```python
from build123d import *

# Parameters (mm, degrees)
BOSS_EXTRUDE1_DEPTH   = 210
SKETCH2_OUTSIDE_W     = 58.016
SKETCH2_OUTSIDE_H     = 56.16
SKETCH2_OUTSIDE_R     = 5
CUT_EXTRUDE1_DEPTH    = 8
SKETCH3_OUTSIDE_W     = 58.016
SKETCH3_OUTSIDE_H     = 56.16
SKETCH3_OUTSIDE_R     = 5
CUT_EXTRUDE2_DEPTH    = 8
M6_TAPPED_HOLE1_D     = 5
M5_TAPPED_HOLE1_D     = 4.2
M5_TAPPED_HOLE1_DEPTH = 12.4
M5_TAPPED_HOLE1_TIP   = 1.2618073
M5_TAPPED_HOLE2_D     = 4.2
M5_TAPPED_HOLE2_DEPTH = 12.4
M5_TAPPED_HOLE2_TIP   = 1.2618073
CHAMFER1_SIZE         = 0.3


with BuildPart() as part:
    # Sketch1 → Boss-Extrude1 (new body)
    with BuildSketch(Plane(origin=(0, 0, 0), x_dir=(1, 0, 0), z_dir=(0, 1, 0))):
        Polygon((6.92820323, 0), (3.464101615, 6), (-3.464101615, 6), (-6.92820323, 0), (-3.464101615, -6), (3.464101615, -6), align=None)
    extrude(amount=BOSS_EXTRUDE1_DEPTH)

    # Sketch2 outside → Cut-Extrude1 (cut)
    with BuildSketch(Plane(origin=(0, 210, 0), x_dir=(1, 0, 0), z_dir=(0, 1, 0))):
        Rectangle(SKETCH2_OUTSIDE_W, SKETCH2_OUTSIDE_H)
        with Locations(Location((0, 0, 0), (0, 0, 270))):
            Circle(SKETCH2_OUTSIDE_R, mode=Mode.SUBTRACT)
    extrude(amount=-CUT_EXTRUDE1_DEPTH, mode=Mode.SUBTRACT)

    # Sketch3 outside → Cut-Extrude2 (cut)
    with BuildSketch(Plane.XZ):
        Rectangle(SKETCH3_OUTSIDE_W, SKETCH3_OUTSIDE_H)
        with Locations(Location((0, 0, 0), (0, 0, 90))):
            Circle(SKETCH3_OUTSIDE_R, mode=Mode.SUBTRACT)
    extrude(amount=-CUT_EXTRUDE2_DEPTH, mode=Mode.SUBTRACT)

    # M6 Tapped Hole1 (through all)
    with Locations(Plane(origin=(0, 0, -6), x_dir=(-1, 0, 0), z_dir=(0, 0, -1))):
        with Locations((0, 140), (0, 70)):
            Hole(M6_TAPPED_HOLE1_D / 2)

    # M5 Tapped Hole1
    with Locations(Plane.XZ):
        with Locations((0, 0)):
            Hole(M5_TAPPED_HOLE1_D / 2, depth=M5_TAPPED_HOLE1_DEPTH)
            with Locations((0, 0, -(M5_TAPPED_HOLE1_DEPTH + M5_TAPPED_HOLE1_TIP / 2))):  # 118° drill point
                Cone(0, M5_TAPPED_HOLE1_D / 2, M5_TAPPED_HOLE1_TIP, mode=Mode.SUBTRACT)

    # M5 Tapped Hole2
    with Locations(Plane(origin=(0, 210, 0), x_dir=(-1, 0, 0), z_dir=(0, 1, 0))):
        with Locations((0, 0)):
            Hole(M5_TAPPED_HOLE2_D / 2, depth=M5_TAPPED_HOLE2_DEPTH)
            with Locations((0, 0, -(M5_TAPPED_HOLE2_DEPTH + M5_TAPPED_HOLE2_TIP / 2))):  # 118° drill point
                Cone(0, M5_TAPPED_HOLE2_D / 2, M5_TAPPED_HOLE2_TIP, mode=Mode.SUBTRACT)

    # Chamfer1
    chamfer1_edges = [part.edges().sort_by_distance(p)[0] for p in [
        (0, 210, -5),
        (0, 0, -5),
    ]]
    chamfer(chamfer1_edges, length=CHAMFER1_SIZE)


solid = part.part
```
The model under review builds one solid part; all positions refer to its coordinate system, in mm. A direction names the side the tool comes from. Round coordinates to 2 decimals unless told otherwise and drop trailing zeros. Order: outer loops, then holes, each group sorted by start corner. A loop starts at its lowest first (then second) coordinate and runs counter-clockwise, first axis right, second up. Notation, with made-up numbers: M -37,59 L 21,59 A24 ccw 21,95 Z; hole C 34,37.5 d11. An arc over 180 degrees is marked long. Use a Markdown table: item, result.
1) Consider section A-A (y = 70). Write out the cut boundary in (x, z).
Report:
| item | result |
|---|---|
| outline | M -6.93,0 L -3.46,-6 L -2.5,-6 L -2.5,6 L -3.46,6 Z; M 2.5,-6 L 3.46,-6 L 6.93,0 L 3.46,6 L 2.5,6 Z |
2) Tool access review of faces 1 (the face through (-4.88, 205.9, -1.08)), 2 (the face through (-5.172, 103.642, -3.042)), 3 (the face through (-2.003, 6.287, 0.631)): name each direction out of +Z, -Z, +X, -X, +Y, -Y from which nothing blocks a thin tool from reaching the whole face with its end or side.
Report:
| item | result |
|---|---|
| face 1 | +Y |
| face 2 | -Z, -X, +Y, -Y |
| face 3 | -Y |
3) Draft analysis for pull direction X (two halves, no side actions). For faces 4 (the face through (-0.33, 142.48, 0.08)), 5 (the face through (-1.1, 0, 2)), 6 (the face through (5.172, 103.642, 3.042)), state which applies: released by +X, released by -X, zero draft, split by the parting line, or undercut.
Report:
| item | result |
|---|---|
| face 4 | undercut |
| face 5 | zero draft |
| face 6 | released by +X |
4) Consider section B-B (y = 134). Write out the cut boundary in (x, z), then the cut area to 3 significant figures.
Report:
| item | result |
|---|---|
| outline | M -6.93,0 L -3.46,-6 L 3.46,-6 L 6.93,0 L 3.46,6 L -3.46,6 Z |
| area | 125 mm^2 |
5) Insertion check: pin 1 (1 mm diameter, centred on x = 4.5, y = 138.5, fed in from +Z); pin 2 (4 mm diameter, centred on x = 0, z = 0, fed in from -Y); pin 3 (2 mm diameter, centred on y = 125, z = -1.5, fed in from -X). Each pin has a flat end and moves straight along its axis. Give the tip position at first contact, or say it passes through.
Report:
| item | result |
|---|---|
| pin 1 | z = 5.07 |
| pin 2 | y = 12.46 |
| pin 3 | x = -6.64 |
6) Wall thickness on line 1 along Y through (x, z) = (0, 3.25); line 2 along X through (y, z) = (205, 0); line 3 along X through (y, z) = (8.75, 0): over which ranges is each line inside the solid? List them lowest first. Write a range as [from, to].
Report:
| item | result |
|---|---|
| line 1 | [0, 67.5], [72.5, 137.5], [142.5, 210] |
| line 2 | [-5, -2.1], [2.1, 5] |
| line 3 | [-6.93, -2.1], [2.1, 6.93] |
